For this review, take the finished solid that the model builds, in its own axes (mm). Face numbers are marked on the shaded views. A direction names the side the tool comes from. Coordinates: 2 decimals unless noted, no trailing zeros. Write each loop counter-clockwise with the first axis right and the second up, starting at its lowest first coordinate (ties: lowest second). Pieces come first, ordered by that corner, then holes. Notation, with made-up numbers: (-7, 0.5) -> (11, 0.5) arc R26 cw to (11, 23.5) -> close; hole circle Ø7 at (-10, 10). An arc over 180 degrees is marked (long way). Put each result on its own line as item: value. Start each with the question number.
Item 1: To check wall thickness, follow L1, parallel to Y at x = 0, z = 3; L2, parallel to Y at x = 25, z = 1.1; L3, parallel to X at y = -12.5, z = 0.9. State the ranges of each line that lie inside material, in increasing order.
Item 2: The part is to be moulded in two halves that separate along X. For the marked faces 3, 4 and 5, say which applies: +X half, -X half, draft (parallel to the pull), parting line (faces both ways), or undercut.
Item 3: For the marked faces 1 and 2, list the 3-axis set-ups (+Z, -Z, +X, -X, +Y, -Y) from which the entire face can be reached by the end or side of a thin tool; tool diameter is ignored.
Item 4: Consider section D-D on x = 24.5. Give the boundary of the cut face in (y, z).
Item 5: Consider section A-A on z = 3.15. Give the boundary of the cut face in (x, y), and give its area (3 significant figures).
Item 6: Insertion check: P1, Ø5, axis at x = 9, y = -29.5, coming from the +Z side; P2, Ø2, axis at x = 2, y = -27.5, coming from the -Z side. Each pin has a flat end and moves straight along its axis. Give the tip position at first contact, or say it passes through.
Item 7: Consider section C-C on y = -31.5. Give the boundary of the cut face in (x, z).
Item 8: Consider section B-B on x = -1. Give the boundary of the cut face in (y, z), and give its area (3 significant figures).
```python
from build123d import *

# Parameters (mm, degrees)
L_LINK_PROFILE_R       = 2.5
L_LINK_PLATE_5MM_DEPTH = 5


with BuildPart() as part:
    # L-Link Profile → L-Link Plate 5mm (new body)
    # profile 1 of 3: a face of its own
    with BuildSketch(Plane.XY):
        with BuildLine():
            Line((25, 5), (0, 5))
            ThreePointArc((0, 5), (3.535533906, 3.535533906), (5, 0))
            Line((5, 0), (5, -5))
            Line((5, -5), (25, -5))
            ThreePointArc((25, -5), (30, 0), (25, 5))
        make_face()
        with Locations((25, 0)):
            Circle(L_LINK_PROFILE_R, mode=Mode.SUBTRACT)
    # profile 2 of 3: a face of its own
    with BuildSketch(Plane.XY):
        with BuildLine():
            Line((-5, 0), (-5, -30))
            ThreePointArc((-5, -30), (0, -35), (5, -30))
            Line((5, -30), (5, -5))
            Line((5, -5), (0, -5))
            ThreePointArc((0, -5), (-3.535533906, -3.535533906), (-5, 0))
        make_face()
        with Locations((0, -30)):
            Circle(L_LINK_PROFILE_R, mode=Mode.SUBTRACT)
    # profile 3 of 3: a face of its own
    with BuildSketch(Plane.XY):
        with BuildLine():
            ThreePointArc((0, 5), (-3.535533906, 3.535533906), (-5, 0))
            ThreePointArc((-5, 0), (-3.535533906, -3.535533906), (0, -5))
            Line((0, -5), (5, -5))
            Line((5, -5), (5, 0))
            ThreePointArc((5, 0), (3.535533906, 3.535533906), (0, 5))
        make_face()
        Circle(L_LINK_PROFILE_R, mode=Mode.SUBTRACT)
    extrude(amount=L_LINK_PLATE_5MM_DEPTH)


solid = part.part
```
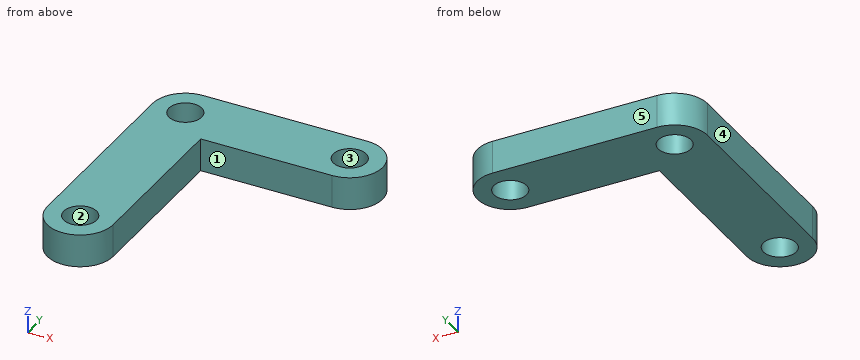
Return value:
1. L1: -35 to -32.5, -27.5 to -2.5, 2.5 to 5
1. L2: -5 to -2.5, 2.5 to 5
1. L3: -5 to 5
2. face 3: undercut
2. face 4: -X half
2. face 5: draft
3. face 1: +Z, -Z, +X, -Y
3. face 2: +Z, -Z
4. outline: (-5, 0) -> (-2.45, 0) -> (-2.45, 5) -> (-5, 5) -> close; (2.45, 0) -> (5, 0) -> (5, 5) -> (2.45, 5) -> close
5. outline: (-5, -30) arc R5 ccw to (5, -30) -> (5, -5) -> (25, -5) arc R5 ccw to (25, 5) -> (0, 5) arc R5 ccw to (-5, 0) -> close; hole circle Ø5 at (0, -30); hole circle Ø5 at (0, 0); hole circle Ø5 at (25, 0)
5. area: 564 mm^2
6. P1: through
6. P2: z = 0
7. outline: (-4.77, 0) -> (-2, 0) -> (-2, 5) -> (-4.77, 5) -> close; (2, 0) -> (4.77, 0) -> (4.77, 5) -> (2, 5) -> close
8. outline: (-34.9, 0) -> (-32.29, 0) -> (-32.29, 5) -> (-34.9, 5) -> close; (-27.71, 0) -> (-2.29, 0) -> (-2.29, 5) -> (-27.71, 5) -> close; (2.29, 0) -> (4.9, 0) -> (4.9, 5) -> (2.29, 5) -> close
8. area: 153 mm^2
